For this review, use the dimensioned drawing (mm, ordinates from the lowest corner) and the shaded views. Coordinates: 2 decimals unless noted, no trailing zeros. Loops run counter-clockwise (first coordinate to the right, second up) from the corner with the lowest first, then second, coordinate; pieces in that order, holes last. Notation, with made-up numbers: M 1,40.25 L 38,40.25 A20 cw 38,77.25 Z; hole C 42,-27 d1. An arc over 180 degrees is marked long. Write each question's results on one line, items separated by ' | '. Start each with the question number.
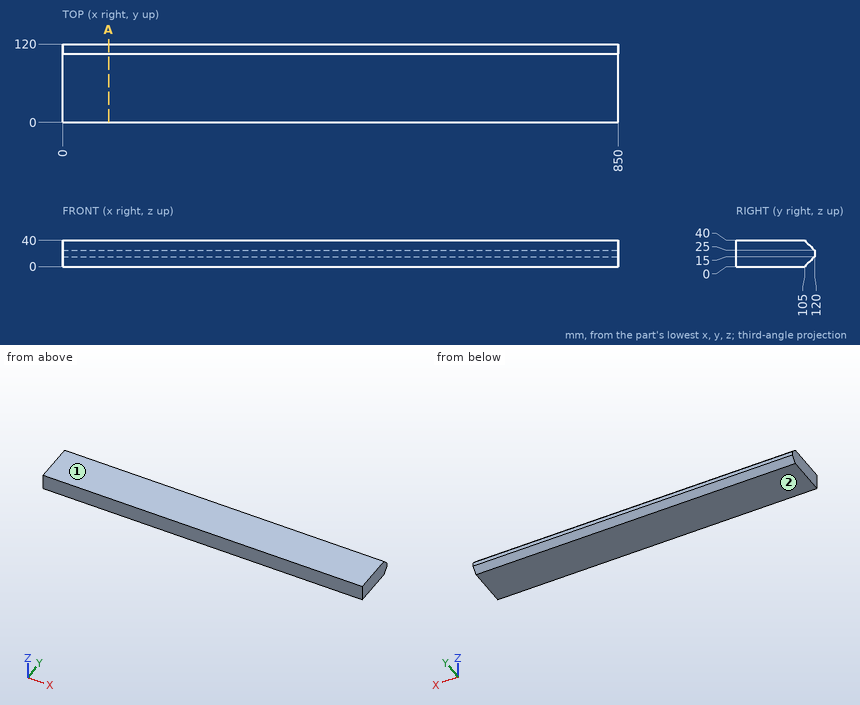
Q1. To check wall thickness, follow line 1 along Y through (x, z) = (239, 7); line 2 along Y through (x, z) = (341, 8); line 3 along Z through (x, y) = (307, 110.5). State the ranges of each line that lie inside material, in increasing order.
Q2. Take a section at A-A, the plane x = 70.5. Give the boundary of the cut face in (y, z).
Q3. The part is to be moulded in two halves that separate along Z. For the marked faces 1 and 2, say which applies: pulls with the +Z half, pulls with the -Z half, needs draft (parallel to the pull), parting line crosses it, or undercut.
Results:
1) line 1: 0 to 112 | line 2: 0 to 113 | line 3: 5.5 to 34.5
2) outline: M 0,0 L 105,0 L 120,15 L 120,25 L 105,40 L 0,40 Z
3) face 1: pulls with the +Z half | face 2: pulls with the -Z half
